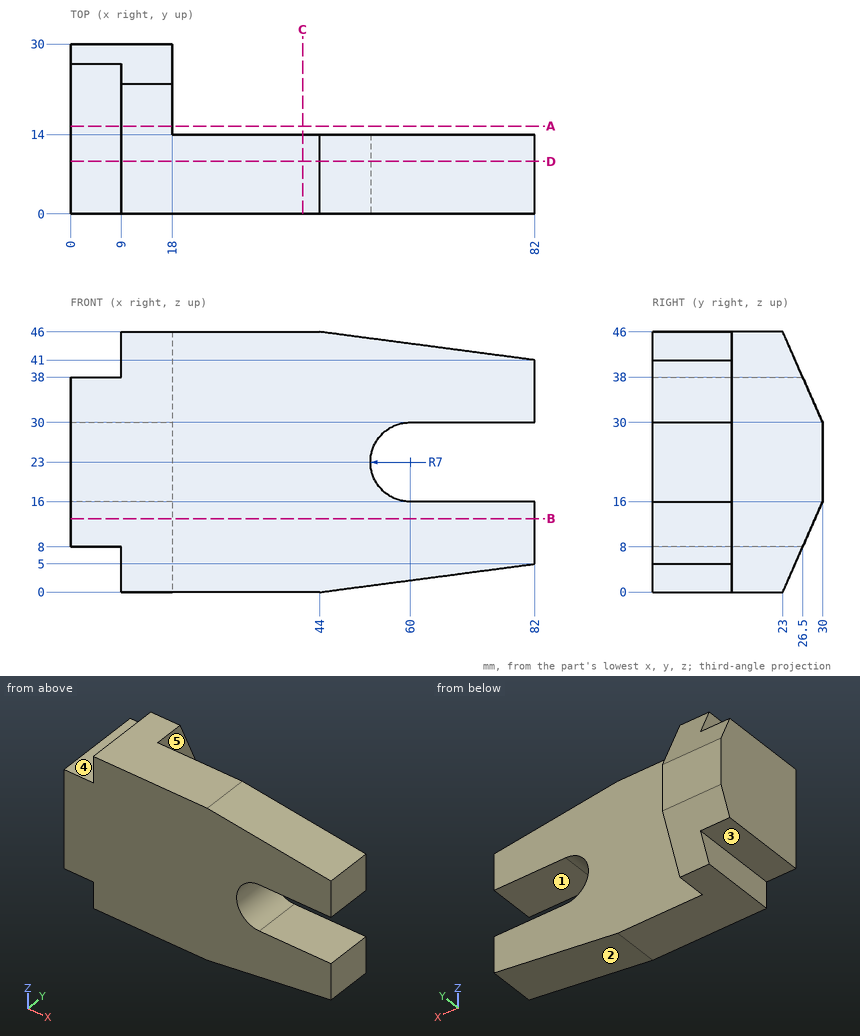
Input: dimensioned drawing with shaded views. Units: mm. Origin: part minimum x, y, z. A direction names the side the tool comes from. Round coordinates to 2 decimals unless told otherwise and drop trailing zeros. Order: outer loops, then holes, each group sorted by start corner. A loop starts at its lowest first (then second) coordinate and runs counter-clockwise, first axis right, second up.
1. Cut plane D-D, the plane y = 9.25. Output: boundary loops of the cut face in (x, z).
The answers:
outline: (0, 8) - (9, 8) - (9, 0) - (44, 0) - (82, 5) - (82, 16) - (60, 16) arc R7 cw to (60, 30) - (82, 30) - (82, 41) - (44, 46) - (9, 46) - (9, 38) - (0, 38) - close
2. Cut plane B-B, the plane z = 13. Output: boundary loops of the cut face in (x, y), then the cut area to 3 significant figures.
The answers:
outline: (0, 0) - (82, 0) - (82, 14) - (18, 14) - (18, 28.69) - (0, 28.69) - close
area: 1,410 mm2
3. Pin query (flat end, axial travel): P1, Ø15.5, axis at x = 66.5, y = 10, coming from the -Z side; P2, Ø10, axis at x = 2.5, y = 16, coming from the -Z side; P3, Ø4, axis at x = 72.5, y = 8, coming from the +Z side. Return the tip coordinate at first contact, or that it passes through.
The answers:
P1: stops at z = 1.94
P2: stops at z = 8
P3: stops at z = 42.51
4. Set-up query: the marked faces 1, 2, 3, 4 and 5. Return all of +Z, -Z, +X, -X, +Y, -Y with unobstructed straight access to the full face (end or side cutting, diameter ignored); none if empty.
The answers:
face 1: +X, +Y, -Y
face 2: -Z, +X, +Y, -Y
face 3: -Z, -X, +Y, -Y
face 4: +Z, -X, +Y, -Y
face 5: +Z, -Z, +X, +Y
5. Cut plane C-C, the plane x = 41. Output: boundary loops of the cut face in (y, z).
The answers:
outline: (0, 0) - (14, 0) - (14, 46) - (0, 46) - close
6. Cut plane A-A, the plane y = 15.5. Output: boundary loops of the cut face in (x, z).
The answers:
outline: (0, 8) - (9, 8) - (9, 0) - (18, 0) - (18, 46) - (9, 46) - (9, 38) - (0, 38) - close
7. Material intervals for line 1 (Y direction, x = 52.5, z = 31.5); line 2 (X direction, y = 15.5, z = 23.5); line 3 (X direction, y = 14.75, z = 39), sorted ascending.
The answers:
line 1: y = 0 to 14
line 2: x = 0 to 18
line 3: x = 9 to 18
